Build history of the part. All positions in model axes, mm. Face numbers are marked on the shaded views. A direction names the side the tool comes from. Give positions to 0.01 mm unless a question says otherwise; leave off trailing zeros. Loops run counter-clockwise (first coordinate to the right, second up) from the corner with the lowest first, then second, coordinate; pieces in that order, holes last.
1) Band-saw the part on B-B on y = -45. List the corners of the cut face in (x, z).
2) Two-plate mould, pull along Y, no slides. Class the marked faces 5, 6 and 7: +Y half, -Y half, draft (parallel to the pull), parting line (faces both ways), or undercut.
3) Band-saw the part on C-C on x = 0. List the corners of the cut face in (y, z).
4) 3-axis set-ups, long thin cutter, end or side, ignore diameter. For the marked faces 1, 2, 3 and 4: which of +Z, -Z, +X, -X, +Y, -Y reach the whole face in a straight line?
5) Band-saw the part on D-D on z = 72. List the corners of the cut face in (x, y), then the cut area to 3 significant figures.
6) Band-saw the part on A-A on z = 37. List the corners of the cut face in (x, y), then the cut area to 3 significant figures.
7) Wall check: line 1 (Y direction, x = 0, z = 23.5); line 2 (X direction, y = 45, z = 65.5); line 3 (Z direction, x = -3, y = -61). Give the ranges that are in metal, low to high.
8) Flat gauge pins, fed straight in: P1, Ø23, axis at x = -13.5, y = -9, coming from the +Z side; P2, Ø19, axis at x = -30, y = 8, coming from the -Z side; P3, Ø6, axis at y = -9.5, z = -6.5, coming from the +X side. Where does each tip first touch, or does it go through?
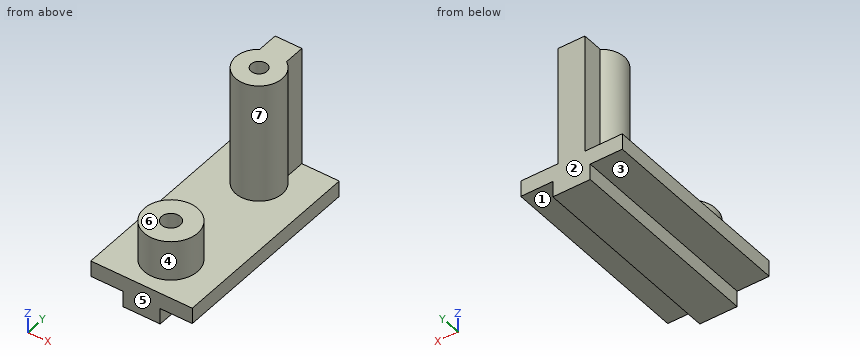
```python
from build123d import *

# Parameters (mm, degrees)
BASE_PLATE_SKETCH_W           = 76
BASE_PLATE_SKETCH_H           = 150
BASE_PLATE_DEPTH              = 12
TOP_TAB_SKETCH_W              = 28
TOP_TAB_SKETCH_H              = 12
TOP_TAB_DEPTH                 = 150
LOWER_BUSHING_BOSS_SKETCH_R   = 20
LOWER_BUSHING_BOSS_SKETCH_R_2 = 7
LOWER_BUSHING_BOSS_DEPTH      = 30
UPPER_ARM_SKETCH_R            = 17.5
UPPER_ARM_SKETCH_R_2          = 6
UPPER_ARM_DEPTH               = 90
ARM_RIB_REACH                 = 187.332
ARM_RIB_END_RADIUS            = 17.5
ARM_RIB_SKETCH_W              = 20
ARM_RIB_SKETCH_H              = 90


with BuildPart() as part:
    # Base Plate Sketch → Base Plate (new body)
    with BuildSketch(Plane.XY):
        Rectangle(BASE_PLATE_SKETCH_W, BASE_PLATE_SKETCH_H)
    extrude(amount=BASE_PLATE_DEPTH)

    # Top Tab Sketch → Top Tab (add, through all)
    with BuildSketch(Plane.XZ.offset(75)):
        with Locations((0, -6)):
            Rectangle(TOP_TAB_SKETCH_W, TOP_TAB_SKETCH_H)
    extrude(amount=-TOP_TAB_DEPTH)

    # Lower Bushing Boss Sketch → Lower Bushing Boss (add)
    with BuildSketch(Plane.XY.offset(12)):
        with Locations(Location((0, -45, 0), (0, 0, 180))):
            Circle(LOWER_BUSHING_BOSS_SKETCH_R)
        with Locations((0, -45)):
            Circle(LOWER_BUSHING_BOSS_SKETCH_R_2, mode=Mode.SUBTRACT)
    extrude(amount=LOWER_BUSHING_BOSS_DEPTH)

    # Upper Arm Sketch → Upper Arm (add)
    with BuildSketch(Plane.XY.offset(12)):
        with Locations(Location((0, 45, 0), (0, 0, 180))):
            Circle(UPPER_ARM_SKETCH_R)
        with Locations(Location((0, 45, 0), (0, 0, 180))):
            Circle(UPPER_ARM_SKETCH_R_2, mode=Mode.SUBTRACT)
    extrude(amount=UPPER_ARM_DEPTH)

    # Arm Rib: up to this cylinder (the profile starts outside it)
    arm_rib_end = Plane(origin=(0, 45, 57), z_dir=(0, 0, -1)) * Cylinder(ARM_RIB_END_RADIUS, 410.664, mode=Mode.PRIVATE)
    # Arm Rib Sketch → Arm Rib (add, up to the surface)
    with BuildSketch(Plane(origin=(0, 75, 0), x_dir=(1, 0, 0), z_dir=(0, 1, 0)), mode=Mode.PRIVATE) as arm_rib_sk1:
        with Locations((0, -57)):
            Rectangle(ARM_RIB_SKETCH_W, ARM_RIB_SKETCH_H)
    arm_rib_tool1 = extrude(arm_rib_sk1.sketch, amount=-ARM_RIB_REACH, mode=Mode.PRIVATE) - arm_rib_end
    add(arm_rib_tool1.solids().sort_by_distance((0, 75, 57))[0])


solid = part.part
```
Findings below:
1. outline: (-38, 0) - (-14, 0) - (-14, -12) - (14, -12) - (14, 0) - (38, 0) - (38, 12) - (20, 12) - (20, 42) - (7, 42) - (7, 12) - (-7, 12) - (-7, 42) - (-20, 42) - (-20, 12) - (-38, 12) - close
2. face 5: -Y half
2. face 6: draft
2. face 7: undercut
3. outline: (-75, -12) - (75, -12) - (75, 102) - (51, 102) - (51, 12) - (39, 12) - (39, 102) - (27.5, 102) - (27.5, 12) - (-25, 12) - (-25, 42) - (-38, 42) - (-38, 12) - (-52, 12) - (-52, 42) - (-65, 42) - (-65, 12) - (-75, 12) - close
4. face 1: -Z, +X, +Y, -Y
4. face 2: +Z, -Z, +X, -X, +Y
4. face 3: -Z, -X, +Y, -Y
4. face 4: +Z
5. outline: (-10, 59.36) arc R17.5 ccw (long way) to (10, 59.36) - (10, 75) - (-10, 75) - close; hole circle Ø12 at (0, 45)
5. area: 1,120 mm2
6. outline: circle Ø40 at (0, -45); (-10, 59.36) arc R17.5 ccw (long way) to (10, 59.36) - (10, 75) - (-10, 75) - close; hole circle Ø14 at (0, -45); hole circle Ø12 at (0, 45)
6. area: 2,220 mm2
7. line 1: y = -65 to -52, -38 to -25, 27.5 to 39, 51 to 75
7. line 2: x = -17.5 to -6, 6 to 17.5
7. line 3: z = -12 to 42
8. P1: stops at z = 12
8. P2: stops at z = 0
8. P3: stops at x = 14
